Read the model definition and answer for the solid it produces. Units are mm, in the model's axes. A direction names the side the tool comes from. Round coordinates to 2 decimals unless told otherwise and drop trailing zeros. Write each loop counter-clockwise with the first axis right and the second up, starting at its lowest first coordinate (ties: lowest second). Pieces come first, ordered by that corner, then holes.
from build123d import *


with BuildPart() as part:
    # 草图1 → 旋转1 (revolve)
    with BuildSketch(Plane.XY, mode=Mode.PRIVATE) as revolve_1_sk:
        Polygon((-37, 0), (-37, 2), (-40, 2), (-40, 15), (-48, 15), (-48, 13.5), (-43, 13.5), (-43, 0), align=None)
    revolve(revolve_1_sk.sketch.rotate(Axis((0, 0, 0), (0, 1, 0)), 270), axis=Axis((0, 0, 0), (0, 1, 0)))


solid = part.part
Q1. Determine the mould class of faces 4 (the cylindrical face through (14.17, 1.01, -34.18)), 5 (the flat face through (-36, 15, -18)), 6 (the cylindrical face through (-14.418, 14.24, -45.783)) for opening direction Z: pulls with the +Z half, pulls with the -Z half, needs draft (parallel to the pull), parting line crosses it, or undercut.
Verdict:
face 4: undercut
face 5: needs draft
face 6: parting line crosses it
Q2. Which of the six approach directions +Z, -Z, +X, -X, +Y, -Y give full straight-line access (tool end or side, diameter ignored) to faces 1 (the flat face through (-18, 13.5, 39.3)), 2 (the cylindrical face through (39.05, 8.59, 8.67)), 3 (the flat face through (-32, 0, -19))?
Verdict:
face 1: -Y
face 2: +Y
face 3: +Z, -Z, +X, -X, -Y
Q3. Flat-ended cylindrical pins translate along their axes: pin 1 Ø8 at (x, y) = (30.5, 5) entering from +Z; pin 2 Ø8 at (y, z) = (12.5, 6) entering from -X; pin 3 Ø5 at (x, y) = (-2, 4) entering from -Z; pin 4 Ø6 at (x, z) = (37, 14.5) entering from -Y. Find the tip coordinate at first contact, or state that the pin passes through.
Verdict:
pin 1: stops at z = 33.86
pin 2: stops at x = -47.95
pin 3: stops at z = -43
pin 4: stops at y = 0
Q4. Straight lines are drawn through the part: probe 1 along X at (y, z) = (10.75, 0); probe 2 along X at (y, z) = (1.35, 0); probe 3 along Y at (x, z) = (26, 35). For each, find the intervals that lie inside material, in ascending order.
Verdict:
probe 1: x = -43 to -40, 40 to 43
probe 2: x = -43 to -37, 37 to 43
probe 3: y = 13.5 to 15
Q5. Section A-A (x = 31) is taken. Determine the outline of the cut face in (y, z), then the cut area to 3 significant figures.
Verdict:
outline: (0, -29.8) - (13.5, -29.8) - (13.5, -36.65) - (15, -36.65) - (15, -25.28) - (2, -25.28) - (2, -20.2) - (0, -20.2) - close; (0, 20.2) - (2, 20.2) - (2, 25.28) - (15, 25.28) - (15, 36.65) - (13.5, 36.65) - (13.5, 29.8) - (0, 29.8) - close
area: 176 mm2
Q6. Section C-C (y = 9.25) is taken. Determine the outline of the cut face in (x, z).
Verdict:
outline: circle Ø86 at (0, 0); hole circle Ø80 at (0, 0)
Q7. Section B-B (z = 0) is taken. Determine the outline of the cut face in (x, y).
Verdict:
outline: (-48, 13.5) - (-43, 13.5) - (-43, 0) - (-37, 0) - (-37, 2) - (-40, 2) - (-40, 15) - (-48, 15) - close; (37, 0) - (43, 0) - (43, 13.5) - (48, 13.5) - (48, 15) - (40, 15) - (40, 2) - (37, 2) - close
Q8. Section D-D (z = 38.5) is taken. Determine the outline of the cut face in (x, y), then the cut area to 3 significant figures.
Verdict:
outline: (-28.67, 13.5) - (-19.15, 13.5) - (-19.15, 0) - (19.15, 0) - (19.15, 13.5) - (28.67, 13.5) - (28.67, 15) - (10.85, 15) - (10.85, 2) - (-10.85, 2) - (-10.85, 15) - (-28.67, 15) - close
area: 321 mm2
